Read the model definition and answer for the solid it produces. Units are mm, in the model's axes. Face numbers are marked on the shaded views. A direction names the side the tool comes from. Give positions to 0.01 mm unless a question says otherwise; leave off trailing zeros. Order: outer loops, then holes, each group sorted by start corner. A loop starts at its lowest first (then second) coordinate and runs counter-clockwise, first axis right, second up. Notation, with made-up numbers: (-11, 87.25) - (5, 87.25) arc R19 cw to (5, 122.25) - close; hole circle Ø5 at (-10, 43). An arc over 180 degrees is marked (long way). Use a Markdown table: item, result. Add a question column.
1. A cutting plane is placed at A-A on z = 0. Determine the outline of the cut face in (x, y), and give its area (3 significant figures).
2. Consider L1, parallel to Z at x = 8.25, y = -0.1; L2, parallel to X at y = 2.2, z = -0.65. Determine where each line is inside the solid, lowest interval first.
3. A cutting plane is placed at C-C on x = 12. Determine the outline of the cut face in (y, z), and give its area (3 significant figures).
4. Which of the six approach directions +Z, -Z, +X, -X, +Y, -Y give full straight-line access (tool end or side, diameter ignored) to the marked faces 1 and 2?
5. A cutting plane is placed at B-B on y = 0. Determine the outline of the cut face in (x, z).
6. Flat-ended cylindrical pins translate along their axes: P1, Ø1.5, axis at x = 19, z = -2, coming from the -Y side; P2, Ø3, axis at x = 18.5, z = -1, coming from the +Y side; P3, Ø1, axis at x = 4.5, z = -1, coming from the +Y side. Find the tip coordinate at first contact, or state that the pin passes through.
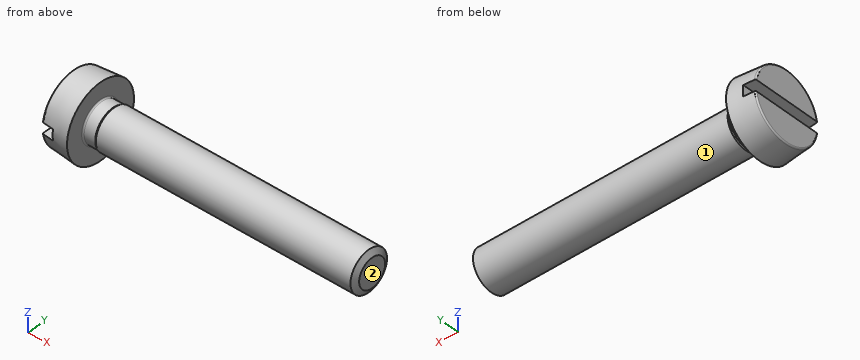
```python
from build123d import *

# Parameters (mm, degrees)
CUT_EXTRUDE1_DEPTH = 0.85


with BuildPart() as part:
    # Sketch1 → Base-Revolve (revolve)
    with BuildSketch(Plane.XY, mode=Mode.PRIVATE) as base_revolve_sk:
        with BuildLine():
            Line((0, 0), (0, 2.483389556))
            ThreePointArc((0, 2.483389556), (0.026272266, 2.550948576), (0.091284426, 2.583009025))
            Line((0.091284426, 2.583009025), (2, 2.75))
            Line((2, 2.75), (2, 1.55))
            ThreePointArc((2, 1.55), (2.029289322, 1.479289322), (2.1, 1.45))
            Line((2.1, 1.45), (2.91339746, 1.45))
            Line((2.91339746, 1.45), (3, 1.5))
            Line((3, 1.5), (22, 1.5))
            Line((22, 1.5), (22, 0))
            Line((22, 0), (0, 0))
        make_face()
    revolve(base_revolve_sk.sketch.rotate(Axis((0, 0, 0), (1, 0, 0)), 90), axis=Axis((0, 0, 0), (1, 0, 0)))

    # Sketch2 → Cut-Extrude1 (cut)
    with BuildSketch(Plane.ZY):
        with BuildLine():
            Line((0.4, 2.720753572), (0.4, -2.720753572))
            ThreePointArc((0.4, -2.720753572), (0, -2.75), (-0.4, -2.720753572))
            Line((-0.4, -2.720753572), (-0.4, 2.720753572))
            ThreePointArc((-0.4, 2.720753572), (0, 2.75), (0.4, 2.720753572))
        make_face()
    extrude(amount=-CUT_EXTRUDE1_DEPTH, mode=Mode.SUBTRACT)

    # Sketch3 → Cut-Revolve1 (revolve, cut)
    with BuildSketch(Plane(origin=(0, 0, 0), x_dir=(1, 0, 0), z_dir=(0, 1, 0)), mode=Mode.PRIVATE) as cut_revolve1_sk:
        Polygon((21.750007333, 1.5), (22.249992667, 1.5), (22, 1.067), align=None)
    revolve(cut_revolve1_sk.sketch.rotate(Axis((0, 0, 0), (1, 0, 0)), 180), axis=Axis((0, 0, 0), (1, 0, 0)), mode=Mode.SUBTRACT)


solid = part.part
```
Output values:
| question | item | result |
|---|---|---|
| 1 | outline | (0.85, -2.65) - (2, -2.75) - (2, -1.55) arc R0.1 cw to (2.1, -1.45) - (2.91, -1.45) - (3, -1.5) - (21.75, -1.5) - (22, -1.07) - (22, 1.07) - (21.75, 1.5) - (3, 1.5) - (2.91, 1.45) - (2.1, 1.45) arc R0.1 cw to (2, 1.55) - (2, 2.75) - (0.85, 2.65) - close |
| 1 | area | 66.0 mm² |
| 2 | L1 | -1.5 to 1.5 |
| 2 | L2 | 0 to 2 |
| 3 | outline | circle Ø3 at (0, 0) |
| 3 | area | 7.07 mm² |
| 4 | face 1 | +X |
| 4 | face 2 | +Z, -Z, +X, +Y, -Y |
| 5 | outline | (0, -2.48) arc R0.1 ccw to (0.09, -2.58) - (2, -2.75) - (2, -1.55) arc R0.1 cw to (2.1, -1.45) - (2.91, -1.45) - (3, -1.5) - (21.75, -1.5) - (22, -1.07) - (22, 1.07) - (21.75, 1.5) - (3, 1.5) - (2.91, 1.45) - (2.1, 1.45) arc R0.1 cw to (2, 1.55) - (2, 2.75) - (0.09, 2.58) arc R0.1 ccw to (0, 2.48) - (0, 0.4) - (0.85, 0.4) - (0.85, -0.4) - (0, -0.4) - close |
| 6 | P1 | y = -0.83 |
| 6 | P2 | y = 1.5 |
| 6 | P3 | y = 1.41 |
